Part model, mm, in its own coordinate system. Give positions to 0.01 mm unless a question says otherwise; leave off trailing zeros. Order: outer loops, then holes, each group sorted by start corner. A loop starts at its lowest first (then second) coordinate and runs counter-clockwise, first axis right, second up.
from build123d import *

# Parameters (mm, degrees)
EXTRUDE_1_DEPTH     = 280
SKETCH_2_R          = 2.5
CUT_EXTRUDE_1_DEPTH = 280
SKETCH_3_R          = 27.5
CUT_EXTRUDE_5_DEPTH = 283.433889606


with BuildPart() as part:
    # 草图1 → 凸台-拉伸1 (new body)
    with BuildSketch(Plane.XY):
        Polygon((0, 0), (0, -3), (37.5, -3), (26.303847577, 0), align=None)
    extrude(amount=EXTRUDE_1_DEPTH)

    # 草图2 → 切除-拉伸1 (cut)
    with BuildSketch(Plane(origin=(0, 0, 0), x_dir=(1, 0, 0), z_dir=(0, 1, 0))):
        with Locations(Location((7.5, -260, 0), (0, 0, 180))):
            Circle(SKETCH_2_R)
        with Locations(Location((7.5, -240, 0), (0, 0, 180))):
            Circle(SKETCH_2_R)
        with Locations(Location((7.5, -20, 0), (0, 0, 180))):
            Circle(SKETCH_2_R)
        with Locations(Location((7.5, -40, 0), (0, 0, 180))):
            Circle(SKETCH_2_R)
    extrude(amount=-CUT_EXTRUDE_1_DEPTH, mode=Mode.SUBTRACT)

    # 草图3 → 切除-拉伸5 (cut, through all)
    with BuildSketch(Plane(origin=(1.762023679, 6.575961894, 0), x_dir=(0.96592582628907, -0.2588190451025147, 0), z_dir=(0.25881904510251463, 0.9659258262890699, 0))):
        with Locations((36.998675621, -140)):
            Circle(SKETCH_3_R)
    extrude(amount=-CUT_EXTRUDE_5_DEPTH, mode=Mode.SUBTRACT)


solid = part.part
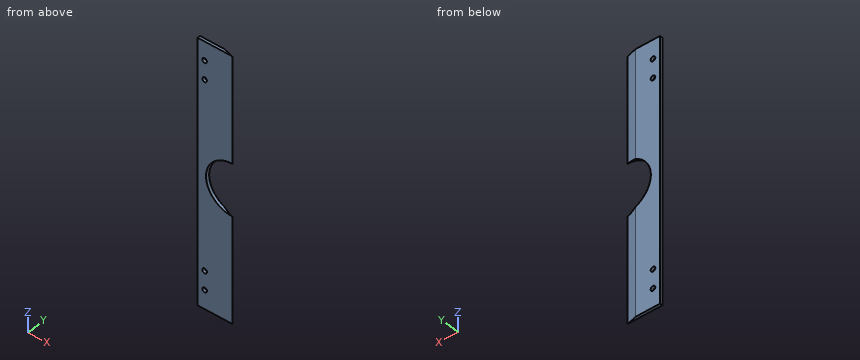
Item 1: Band-saw the part on B-B on z = 139. List the corners of the cut face in (x, y), plus the area to 3 significant figures.
Item 2: Drill centre lines: probe 1 along Z at (x, y) = (7.5, -2.05); probe 2 along Z at (x, y) = (26, -1.55); probe 3 along Z at (x, y) = (7, -1.1). Where is each one in solid material? Low to high.
Item 3: Band-saw the part on C-C on y = -1.65. Give the number of separate pieces and of enclosed holes in the cut face, plus the area to 3 significant figures.
Item 4: Band-saw the part on A-A on z = 40. List the corners of the cut face in (x, y), plus the area to 3 significant figures.
Item 5: Drop a flat-ended pin along its axis: P1, Ø6, axis at x = 7.5, z = 40, coming from the +Y side. Give the stop position or say it passes through.
Working result:
1. outline: (0, -3) - (9.05, -3) - (9.85, 0) - (0, 0) - close
1. area: 28.4 mm2
2. probe 1: z = 0 to 17.5, 22.5 to 37.5, 42.5 to 237.5, 242.5 to 257.5, 262.5 to 280
2. probe 2: z = 0 to 115.01, 164.99 to 280
2. probe 3: z = 0 to 17.55, 22.45 to 37.55, 42.45 to 237.55, 242.45 to 257.55, 262.45 to 280
3. separate pieces: 1
3. enclosed holes: 4
3. area: 8,080 mm2
4. outline: (0, -3) - (5, -3) - (5, 0) - (0, 0) - close; (10, -3) - (37.5, -3) - (26.3, 0) - (10, 0) - close
4. area: 80.7 mm2
5. P1: stops at y = 0
